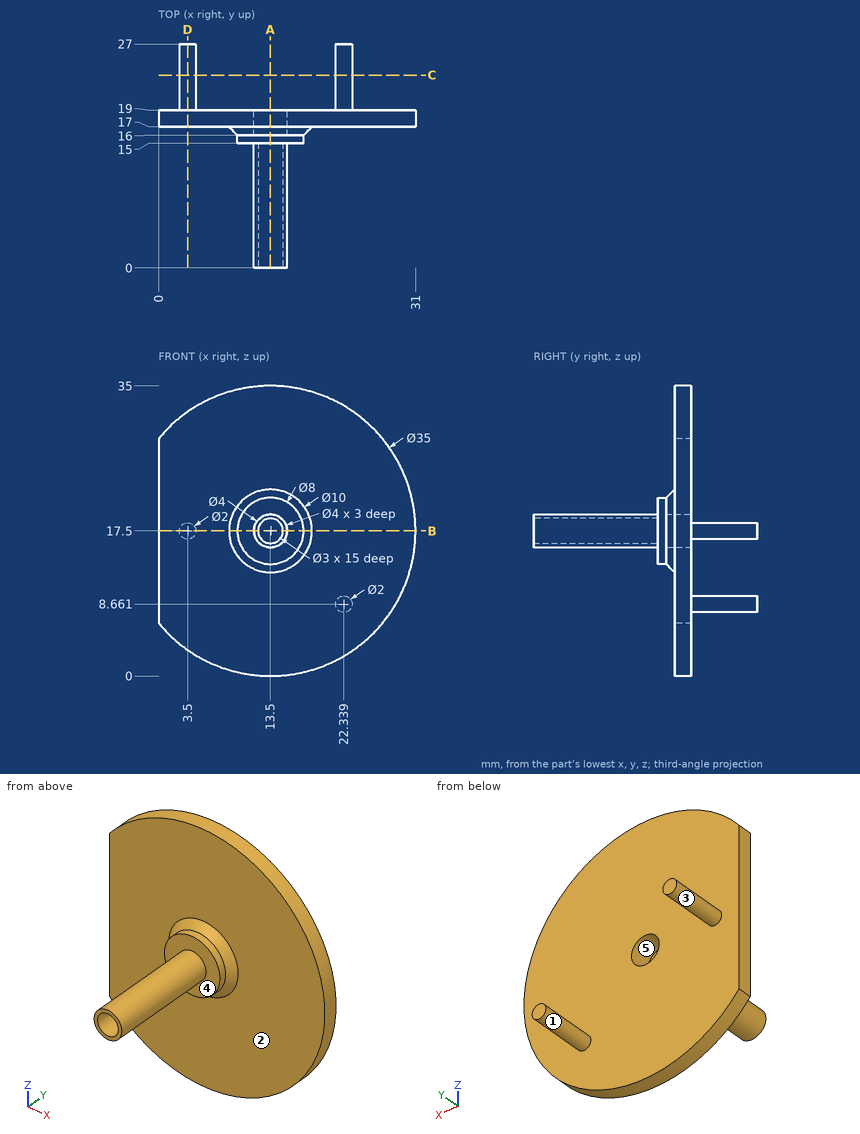
Geometry: see drawing. Coordinates: mm, zero at the bounding-box minimum. A direction names the side the tool comes from. Coordinates: 2 decimals unless noted, no trailing zeros. Loops run counter-clockwise (first coordinate to the right, second up) from the corner with the lowest first, then second, coordinate; pieces in that order, holes last.
(1) First-contact query: pin 1 Ø3 at (x, z) = (17.5, 17.5) entering from -Y; pin 2 Ø1 at (x, z) = (21.5, 13) entering from -Y; pin 3 Ø4 at (x, z) = (18, 12.5) entering from -Y; pin 4 Ø12 at (x, y) = (25, 4) entering from +Z. Flat tips, straight axial feed; report the tip coordinate or a pass-through.
(2) Set-up query: the marked faces 1 and 2. Return all of +Z, -Z, +X, -X, +Y, -Y with unobstructed straight access to the full face (end or side cutting, diameter ignored); none if empty.
(3) Section B-B on z = 17.5. Return the cut outline in (x, y).
(4) Section C-C on y = 23.25. Return the cut outline in (x, z).
(5) Section D-D on x = 3.5. Return the cut outline in (y, z).
(6) Material intervals for probe 1 along X at (y, z) = (18.3, 17.5); probe 2 along Y at (x, z) = (10.5, 10); probe 3 along X at (y, z) = (16.85, 17.5), sorted ascending.
(7) Section A-A on x = 13.5. Return the cut outline in (y, z).
(8) Pull-direction query (X, two-part tool) for the marked faces 3, 4 and 5; classes: released by +X, released by -X, zero draft, split by the parting line, or undercut.
Data:
1. pin 1: stops at y = 15
1. pin 2: stops at y = 17
1. pin 3: stops at y = 16.73
1. pin 4: passes through
2. face 1: +Y
2. face 2: -Y
3. outline: (0, 17) - (8.5, 17) - (9.5, 16) - (9.5, 15) - (11.5, 15) - (11.5, 0) - (12, 0) - (12, 15) - (15, 15) - (15, 0) - (15.5, 0) - (15.5, 15) - (17.5, 15) - (17.5, 16) - (18.5, 17) - (31, 17) - (31, 19) - (15.5, 19) - (15.5, 16) - (11.5, 16) - (11.5, 19) - (4.5, 19) - (4.5, 27) - (2.5, 27) - (2.5, 19) - (0, 19) - close
4. outline: circle Ø2 at (3.5, 17.5); circle Ø2 at (22.34, 8.66)
5. outline: (17, 3.14) - (19, 3.14) - (19, 16.5) - (27, 16.5) - (27, 18.5) - (19, 18.5) - (19, 31.86) - (17, 31.86) - close
6. probe 1: x = 0 to 11.5, 15.5 to 31
6. probe 2: y = 17 to 19
6. probe 3: x = 8.65 to 11.5, 15.5 to 18.35
7. outline: (0, 15.5) - (15, 15.5) - (15, 13.5) - (16, 13.5) - (17, 12.5) - (17, 0) - (19, 0) - (19, 15.5) - (16, 15.5) - (16, 19.5) - (19, 19.5) - (19, 35) - (17, 35) - (17, 22.5) - (16, 21.5) - (15, 21.5) - (15, 19.5) - (0, 19.5) - (0, 19) - (15, 19) - (15, 16) - (0, 16) - close
8. face 3: split by the parting line
8. face 4: zero draft
8. face 5: undercut
